Part model, mm, in its own coordinate system. A direction names the side the tool comes from. Coordinates: 2 decimals unless noted, no trailing zeros. Write each loop counter-clockwise with the first axis right and the second up, starting at its lowest first coordinate (ties: lowest second). Pieces come first, ordered by that corner, then holes. Notation, with made-up numbers: (-0.75, -22.5) -> (37.25, -22.5) arc R6 cw to (37.25, -13.5) -> close; hole circle Ø4 at (86, 77.25). An arc over 180 degrees is marked (long way). Write item = value, one per line.
from build123d import *

# Parameters (mm, degrees)
SKETCH_5_R               = 20.566311538
CUT_EXTRUDE_1_DEPTH      = 0.5
SKETCH_6_R               = 21.52826295
CUT_EXTRUDE_2_DEPTH      = 0.5
EXTRUDE_START            = 11
SKETCH_7_R               = 8.5
SKETCH_7_R_2             = 4
EXTRUDE_1_DEPTH          = 11
SKETCH_10_R              = 15
CUT_EXTRUDE_3_DEPTH      = 15
SKETCH_11_R              = 15
SKETCH_11_R_2            = 4
EXTRUDE_2_DEPTH          = 0.5
EXTRUDE_START_2          = 0.5
SKETCH_12_R              = 15
SKETCH_12_R_2            = 4
EXTRUDE_3_DEPTH          = 0.5
EXTRUDE_START_3          = 8
SKETCH_14_R              = 7
SKETCH_14_R_2            = 4
EXTRUDE_5_DEPTH          = 8
SKETCH_17_R              = 17.215216586
CUT_EXTRUDE_4_DEPTH      = 30.849623113
SKETCH_18_R              = 9
SKETCH_18_R_2            = 4
EXTRUDE_6_DEPTH          = 8
CHAMFER_1_SIZE           = 1
CHAMFER_1_SIZE2          = 0.577350269
CHAMFER_2_SIZE           = 1
CHAMFER_2_SIZE2          = 0.577350269
CHAMFER_3_SIZE           = 0.5
EXTRUDE_8_DEPTH          = 29
SKETCH_19_W              = 1.65
SKETCH_19_H              = 15
PATTERN_CIRCULAR_1_COUNT = 2
PATTERN_CIRCULAR_1_ANGLE = 90
SKETCH_22_R              = 11.227915354
CUT_EXTRUDE_5_DEPTH      = 5
CHAMFER_4_SIZE           = 1
CHAMFER_4_SIZE2          = 0.577350269


with BuildPart() as part:
    # 草图1 → 旋转1 (revolve)
    with BuildSketch(Plane.XY, mode=Mode.PRIVATE) as revolve_1_sk:
        Polygon((4, 0), (4, 21), (15, 21), (15, 19), (12.99, 19), (12.99, 2), (15, 2), (15, 0), align=None)
    revolve(revolve_1_sk.sketch.rotate(Axis((0, 0, 0), (0, 1, 0)), 90), axis=Axis((0, 0, 0), (0, 1, 0)))

    # 草图5 → 切除-拉伸1 (cut)
    with BuildSketch(Plane.XZ):
        Circle(SKETCH_5_R)
    extrude(amount=-CUT_EXTRUDE_1_DEPTH, mode=Mode.SUBTRACT)

    # 草图6 → 切除-拉伸2 (cut)
    with BuildSketch(Plane(origin=(0, 21, 0), x_dir=(1, 0, 0), z_dir=(0, 1, 0))):
        Circle(SKETCH_6_R)
    extrude(amount=-CUT_EXTRUDE_2_DEPTH, mode=Mode.SUBTRACT)

    # 草图7 → 凸台-拉伸1 (add)
    with BuildSketch(Plane(origin=(0, 20.5, 0), x_dir=(1, 0, 0), z_dir=(0, 1, 0)).offset(EXTRUDE_START)):
        with Locations(Location((0, 0, 0), (0, 0, 270))):
            Circle(SKETCH_7_R)
        with Locations(Location((0, 0, 0), (0, 0, 90))):
            Circle(SKETCH_7_R_2, mode=Mode.SUBTRACT)
    extrude(amount=-EXTRUDE_1_DEPTH)

    # 草图10 → 切除-拉伸3 (cut)
    with BuildSketch(Plane(origin=(0, 20.5, 0), x_dir=(1, 0, 0), z_dir=(0, 1, 0))):
        with Locations(Location((0, 0, 0), (0, 0, 90))):
            Circle(SKETCH_10_R)
    extrude(amount=CUT_EXTRUDE_3_DEPTH, mode=Mode.SUBTRACT)

    # 草图11 → 凸台-拉伸2 (add)
    with BuildSketch(Plane(origin=(0, 20.5, 0), x_dir=(1, 0, 0), z_dir=(0, 1, 0))):
        with Locations(Location((0, 0, 0), (0, 0, 90))):
            Circle(SKETCH_11_R)
        with Locations(Location((0, 0, 0), (0, 0, 90))):
            Circle(SKETCH_11_R_2, mode=Mode.SUBTRACT)
    extrude(amount=EXTRUDE_2_DEPTH)

    # 草图12 → 凸台-拉伸3 (add)
    with BuildSketch(Plane.XZ.offset(-0.5).offset(EXTRUDE_START_2)):
        with Locations(Location((0, 0, 0), (0, 0, 270))):
            Circle(SKETCH_12_R)
        with Locations(Location((0, 0, 0), (0, 0, 270))):
            Circle(SKETCH_12_R_2, mode=Mode.SUBTRACT)
    extrude(amount=-EXTRUDE_3_DEPTH)

    # 草图14 → 凸台-拉伸5 (add)
    with BuildSketch(Plane(origin=(0, 21, 0), x_dir=(1, 0, 0), z_dir=(0, 1, 0)).offset(EXTRUDE_START_3)):
        with Locations(Location((0, 0, 0), (0, 0, 270))):
            Circle(SKETCH_14_R)
        with Locations(Location((0, 0, 0), (0, 0, 90))):
            Circle(SKETCH_14_R_2, mode=Mode.SUBTRACT)
    extrude(amount=-EXTRUDE_5_DEPTH)

    # 草图17 → 切除-拉伸4 (cut, through all)
    with BuildSketch(Plane(origin=(0, 21, 0), x_dir=(1, 0, 0), z_dir=(0, 1, 0))):
        Circle(SKETCH_17_R)
    extrude(amount=CUT_EXTRUDE_4_DEPTH, mode=Mode.SUBTRACT)

    # 草图18 → 凸台-拉伸6 (add)
    with BuildSketch(Plane(origin=(0, 21, 0), x_dir=(1, 0, 0), z_dir=(0, 1, 0)).offset(EXTRUDE_START_3)):
        with Locations(Location((0, 0, 0), (0, 0, 270))):
            Circle(SKETCH_18_R)
        with Locations(Location((0, 0, 0), (0, 0, 90))):
            Circle(SKETCH_18_R_2, mode=Mode.SUBTRACT)
    extrude(amount=-EXTRUDE_6_DEPTH)

    # 倒角1
    chamfer_1_edges = [part.edges().sort_by_distance(p)[0] for p in [
        (0, 19, 15),
    ]]
    chamfer_1_side = [part.faces().sort_by_distance(p)[0] for p in [
        (0, 20, 15),
    ]]
    chamfer(chamfer_1_edges, length=CHAMFER_1_SIZE, length2=CHAMFER_1_SIZE2, reference=chamfer_1_side[0])

    # 倒角2
    chamfer_2_edges = [part.edges().sort_by_distance(p)[0] for p in [
        (0, 2, 15),
    ]]
    chamfer_2_side = [part.faces().sort_by_distance(p)[0] for p in [
        (0, 2, 13.414264069),
    ]]
    chamfer(chamfer_2_edges, length=CHAMFER_2_SIZE, length2=CHAMFER_2_SIZE2, reference=chamfer_2_side[0])

    # 倒角3
    chamfer_3_edges = [part.edges().sort_by_distance(p)[0] for p in [
        (0, 29, -9),
    ]]
    chamfer(chamfer_3_edges, length=CHAMFER_3_SIZE)

    # 草图21 → 凸台-拉伸8 (add, through all)
    with BuildSketch(Plane(origin=(0, 29, 0), x_dir=(1, 0, 0), z_dir=(0, 1, 0))):
        with BuildLine():
            Line((-1.936491673, -3.5), (1.936491673, -3.5))
            ThreePointArc((1.936491673, -3.5), (0, -4), (-1.936491673, -3.5))
        make_face()
    extrude(amount=-EXTRUDE_8_DEPTH)

    # 草图19 → M4 螺纹孔1 (revolve, cut)
    with BuildSketch(Plane(origin=(0, 15, 0), x_dir=(0, 1, 0), z_dir=(1, 0, 0))):
        with Locations((0.825, 7.5)):
            Rectangle(SKETCH_19_W, SKETCH_19_H)
    hole_wizard_m4_1 = revolve(axis=Axis((0, 15, -6.35), (0, 0, 1)), mode=Mode.SUBTRACT)

    # 阵列(圆周)1: M4 螺纹孔1 ×2 about axis
    pattern_circular_1_axis = Axis((0, 0, 0), (0, -1, 0))
    for i in range(1, PATTERN_CIRCULAR_1_COUNT):
        add(hole_wizard_m4_1.rotate(pattern_circular_1_axis, i * PATTERN_CIRCULAR_1_ANGLE / (PATTERN_CIRCULAR_1_COUNT - 1)), mode=Mode.SUBTRACT)

    # 草图22 → 切除-拉伸5 (cut)
    with BuildSketch(Plane(origin=(0, 29, 0), x_dir=(1, 0, 0), z_dir=(0, 1, 0))):
        Circle(SKETCH_22_R)
    extrude(amount=-CUT_EXTRUDE_5_DEPTH, mode=Mode.SUBTRACT)

    # 倒角4
    chamfer_4_edges = [part.edges().sort_by_distance(p)[0] for p in [
        (0, 24, -9),
    ]]
    chamfer_4_side = [part.faces().sort_by_distance(p)[0] for p in [
        (0, 22.5, -9),
    ]]
    chamfer(chamfer_4_edges, length=CHAMFER_4_SIZE, length2=CHAMFER_4_SIZE2, reference=chamfer_4_side[0])


solid = part.part
Q1. Probe line 1 (Y direction, x = 4.25, z = -12.5); line 2 (X direction, y = 8.75, z = 0); line 3 (Z direction, x = 3.25, y = 10). List the from-to ranges inside material, lowest first. Write a range as from..to.
Model answer:
line_1 = 0..2, 19..21
line_2 = -12.99..-4, 4..12.99
line_3 = -12.58..-2.33, 2.33..12.58
Q2. Pin check, flat tips, straight feed: pin 1 (5 mm diameter, centred on x = 7.5, y = 19.5, fed in from +Z); pin 2 (4.5 mm diameter, centred on x = 0.5, y = 11.5, fed in from -Z); pin 3 (10 mm diameter, centred on y = 11, z = 9, fed in from +X). Stop position of each tip, or through.
Model answer:
pin_1 = 14.12
pin_2 = -12.99
pin_3 = 12.36
Q3. Saw through at A-A on x = 0. Count the separate pieces of the cut face and the enclosed holes in it, and give its area (3 significant figures).
Model answer:
separate_pieces = 3
enclosed_holes = 0
area = 403 mm²
Q4. Which spindle directions (+Z, -Z, +X, -X, +Y, -Y) get a long thin tool onto all of the face, cutting with end or side? Do faces 1 (the face through (-8.384, 16.574, -0.496)), 2 (the face through (2.703, 22.014, 8.584)), 3 (the face through (9.3, 2, 9.3)). Say none if no direction does.
Model answer:
face_1 = -X
face_2 = +Y
face_3 = none
Q5. Saw through at D-D on y = 6.25. Give the cut face in (x, z).
Model answer:
outline = circle Ø25.98 at (0, 0); hole (-1.94, 3.5) arc R4 ccw (long way) to (1.94, 3.5) -> close
Q6. Mould opens along X. For faces 4 (the face through (-0.496, 16.574, 8.311)), 5 (the face through (-3.9, 10.38, -12.39)), 6 (the face through (6.5, 21, -6.5)) say: released by +X, released by -X, zero draft, split by the parting line, or undercut.
Model answer:
face_4 = undercut
face_5 = split by the parting line
face_6 = zero draft
Q7. Saw through at C-C on y = 15. Give the cut face in (x, z), and give its area (3 significant figures).
Model answer:
outline = (-12.88, -1.65) arc R12.99 ccw (long way) to (1.65, 12.88) -> (1.65, 3.5) -> (1.94, 3.5) arc R4 cw (long way) to (-3.64, -1.65) -> close; (-12.88, 1.65) -> (-3.64, 1.65) arc R4 cw to (-1.94, 3.5) -> (-1.65, 3.5) -> (-1.65, 12.88) arc R12.99 ccw to start
area = 420 mm²
